Source: CAD feature listing. Evaluate the final solid. Frame: model axes, mm. A direction names the side the tool comes from. Round coordinates to 2 decimals unless told otherwise and drop trailing zeros. Order: outer loops, then holes, each group sorted by start corner. A loop starts at its lowest first (then second) coordinate and runs counter-clockwise, first axis right, second up. Notation, with made-up numbers: (14, 84) - (31, 84) arc R10 cw to (31, 92) - close; hole circle Ø1 at (-28.75, -35.5). An arc over 180 degrees is marked (long way). Return JSON: item names as keys, results as strings. Group by question number.
1) Ray query, line 1 (X direction, y = -8.25, z = 0); line 2 (Y direction, x = 14.5, z = -16); line 3 (X direction, y = -10, z = 2.5). Return the intervals inside material, ascending. Write a range as from..to.
2) Access query for faces 1 (the flat face through (-7.77, 11.42, 21.39)), 2 (the cylindrical face through (-14.65, 9.9, -27.4)), 3 (the flat face through (21.076, 4.521, -3.879)), 4 (the flat face through (0, -6, 8.15)). Directions: +Z, -Z, +X, -X, +Y, -Y. A direction counts if a zero-diameter tool reaches every point of the face in a straight line with its end or side. Return the directions, or none.
3) Section B-B, the plane z = 0. Return loops of the section in (x, y), plus the area to 3 significant figures.
4) Section D-D, the plane z = 20. Return loops of the section in (x, y), plus the area to 3 significant figures.
5) Section C-C, the plane x = -28. Return loops of the section in (y, z), plus the area to 3 significant figures.
6) Mould query, pull axis X, two halves, no side actions, for faces 5 (the cylindrical face through (15.13, 9.9, 34.7)), 6 (the flat face through (-5.4, -16, -5.4)), 7 (the cylindrical face through (15.17, 9.9, 27.39)), 8 (the cylindrical face through (-22.4, 9.9, 30.2)). Classes: pulls with the +X half, pulls with the -X half, needs draft (parallel to the pull), parting line crosses it, or undercut.
7) Contact query for flat-ended pins moving along their axis: P1, Ø18, axis at x = 0, z = 0, coming from the -Y side; P2, Ø1, axis at x = -6.5, y = -4.5, coming from the -Z side; P3, Ø4, axis at x = -1, y = -9.5, coming from the -Z side; P4, Ø0.5, axis at y = -2, z = 7.5, coming from the +X side. Output: stop coordinate, or through.
8) Section A-A, the plane x = 0. Return loops of the section in (y, z).
```python
from build123d import *
from build123d.topology import SkipClean

# Parameters (mm, degrees)
BASE_DISC_SKETCH_R                         = 37.5
BASE_DISC_75_DEPTH                         = 3
VANE_DEPTH                                 = 14
VANE_CHAMFER_3MM_SIZE                      = 3
VANE_PATTERN_6X60_COUNT                    = 6
VANE_CHAMFER_3MM_OF_VANE_PATTERN_6X60_SIZE = 3
HUB_SKETCH_R                               = 12.5
HUB_25_DEPTH                               = 16
SHAFT_BORE_14_DEPTH                        = 63.702444686
SHAFT_BORE_14_DEPTH_BACK                   = 63.702444686
HUB_FILLET_R6_R                            = 6


with BuildPart() as part:
    # Base Disc Sketch → Base Disc Ø75 (new body)
    with BuildSketch(Plane(origin=(0, 0, 0), x_dir=(1, 0, 0), z_dir=(0, 1, 0))):
        with Locations(Location((0, 0, 0), (0, 0, 270))):
            Circle(BASE_DISC_SKETCH_R)
    extrude(amount=BASE_DISC_75_DEPTH)

    # Vane Profile Sketch → Vane (add)
    with SkipClean():  # the faces are left unmerged after this step: merging them gives an invalid solid
        with BuildSketch(Plane(origin=(0, 3, 0), x_dir=(1, 0, 0), z_dir=(0, 1, 0))):
            with BuildLine():
                Line((-22.661730354, -3), (-21.896634912, -4.5))
                ThreePointArc((-21.896634912, -4.5), (-30.228522345, -1.968631367), (-37.379807383, 3))
                ThreePointArc((-37.379807383, 3), (-37.228578705, 4.503657138), (-37.016888038, 6))
                ThreePointArc((-37.016888038, 6), (-30.466111276, 0.5002397), (-22.661730354, -3))
            make_face()
        vane = extrude(amount=VANE_DEPTH)

    # Vane Chamfer 3mm
    vane_chamfer_3mm_edges = [part.edges().sort_by_distance(p)[0] for p in [
        (-22.279182633, 3, 3.75),
    ]]
    chamfer(vane_chamfer_3mm_edges, length=VANE_CHAMFER_3MM_SIZE)

    # Vane Pattern 6x60°: Vane ×6 about axis
    with SkipClean():  # the faces are left unmerged after this step: merging them gives an invalid solid
        vane_pattern_6x60_axis = Axis((0.259677898, 0, -0.003858097), (0, 1, 0))
        for i in range(1, VANE_PATTERN_6X60_COUNT):
            add(vane.rotate(vane_pattern_6x60_axis, i * 360 / VANE_PATTERN_6X60_COUNT))

    # Vane Chamfer 3mm of Vane Pattern 6x60°
    vane_chamfer_3mm_of_vane_pattern_6x60_edges = [part.edges().sort_by_distance(p)[0] for p in [
        (-7.758815893, 3, 21.392296743),
        (14.780044637, 3, 17.638438646),
        (22.798538428, 3, -3.757716194),
        (8.278171688, 3, -21.400012937),
        (-14.260688842, 3, -17.64615484),
    ]]
    chamfer(vane_chamfer_3mm_of_vane_pattern_6x60_edges, length=VANE_CHAMFER_3MM_OF_VANE_PATTERN_6X60_SIZE)

    # Hub Sketch → Hub Ø25 (add)
    with SkipClean():  # the faces are left unmerged after this step: merging them gives an invalid solid
        with BuildSketch(Plane.XZ):
            with Locations(Location((0, 0, 0), (0, 0, 270))):
                Circle(HUB_SKETCH_R)
        extrude(amount=HUB_25_DEPTH)

    # Shaft Bore Sketch → Shaft Bore Ø14 (cut, two sides: drawn at the far end of the back side and taken through both)
    with SkipClean():  # the faces are left unmerged after this step: merging them gives an invalid solid
        with BuildSketch(Plane.XZ.offset(16).offset(-SHAFT_BORE_14_DEPTH_BACK)):
            with BuildLine():
                Line((-2.5, 8.15), (2.5, 8.15))
                Line((2.5, 8.15), (2.5, 6.538348415))
                ThreePointArc((2.5, 6.538348415), (0, -7), (-2.5, 6.538348415))
                Line((-2.5, 6.538348415), (-2.5, 8.15))
            make_face()
        extrude(amount=SHAFT_BORE_14_DEPTH + SHAFT_BORE_14_DEPTH_BACK, mode=Mode.SUBTRACT)

    # Hub Fillet R6
    hub_fillet_r6_edges = [part.edges().sort_by_distance(p)[0] for p in [
        (0, 0, 12.5),
    ]]
    fillet(hub_fillet_r6_edges, radius=HUB_FILLET_R6_R)


solid = part.part
```
Geometry check:
{
 "1": {"line 1": "-12.5..-7, 7..12.5", "line 2": "0..3", "line 3": "-12.25..-6.54, 6.54..12.25"},
 "2": {"face 1": "-Z, +Y", "face 2": "+Y", "face 3": "+Z, +Y", "face 4": "+Y, -Y"},
 "3": {"outline": "(-37.5, 0) - (-18.5, 0) arc R6 cw to (-12.5, -6) - (-12.5, -16) - (-7, -16) - (-7, 3) - (-29.64, 3) - (-29.64, 17) - (-33.65, 17) - (-33.65, 3) - (-37.5, 3) - close; (7, -16) - (12.5, -16) - (12.5, -6) arc R6 cw to (18.5, 0) - (37.5, 0) - (37.5, 3) - (34.18, 3) - (34.18, 17) - (30.17, 17) - (30.17, 3) - (7, 3) - close", "area": "487 mm2"},
 "4": {"outline": "(-31.72, 0) - (31.72, 0) - (31.72, 3) - (16.28, 3) - (16.28, 17) - (14.68, 17) - (14.68, 3) - (-5.87, 3) - (-5.87, 4.51) - (-7.28, 4.58) - (-7.28, 3) - (-31.72, 3) - close", "area": "215 mm2"},
 "5": {"outline": "(0, -24.94) - (3, -24.94) - (3, 0.89) - (17, 0.89) - (17, 2.93) - (3, 2.93) - (3, 24.94) - (0, 24.94) - close", "area": "178 mm2"},
 "6": {"face 5": "pulls with the +X half", "face 6": "needs draft", "face 7": "undercut", "face 8": "pulls with the -X half"},
 "7": {"P1": "y = -16", "P2": "z = -11.23", "P3": "z = -12.5", "P4": "x = 12.17"},
 "8": {"outline": "(-16, -12.5) - (-6, -12.5) arc R6 cw to (0, -18.5) - (0, -37.5) - (3, -37.5) - (3, -7) - (-16, -7) - close; (-16, 8.15) - (3, 8.15) - (3, 37.5) - (0, 37.5) - (0, 18.5) arc R6 cw to (-6, 12.5) - (-16, 12.5) - close"}
}
